```python
from build123d import *

# Parameters (mm, degrees)
SKETCH1_W                                            = 50
SKETCH1_H                                            = 10
SKETCH1_W_2                                          = 100
SKETCH1_H_2                                          = 200
BOSS_EXTRUDE1_DEPTH                                  = 100
CUT_EXTRUDE1_DEPTH                                   = 174.205080757
CUT_EXTRUDE1_DEPTH_BACK                              = 174.205080757
SKETCH7_W                                            = 80
SKETCH7_H                                            = 80
CUT_EXTRUDE2_DEPTH                                   = 100
SKETCH8_R                                            = 20
CUT_EXTRUDE3_DEPTH                                   = 20
CSK_FOR_M6_HEXAGON_LOBULAR_SOCKET_RAISED_D           = 6.6
CSK_FOR_M6_HEXAGON_LOBULAR_SOCKET_RAISED_CSINK_D     = 12.8
CSK_FOR_M6_HEXAGON_LOBULAR_SOCKET_RAISED_CSINK_ANGLE = 90
SKETCH13_W                                           = 20
SKETCH13_H                                           = 20
CUT_EXTRUDE4_DEPTH                                   = 10


with BuildPart() as part:
    # Sketch1 → Boss-Extrude1 (new body)
    with BuildSketch(Plane.XY):
        with Locations((-75, -95)):
            Rectangle(SKETCH1_W, SKETCH1_H)
        Rectangle(SKETCH1_W_2, SKETCH1_H_2)
        with Locations((75, -95)):
            Rectangle(SKETCH1_W, SKETCH1_H)
    extrude(amount=BOSS_EXTRUDE1_DEPTH)

    # Sketch5 → Cut-Extrude1 (cut, two sides: drawn at the far end of the back side and taken through both)
    with BuildSketch(Plane(origin=(0, 0, 0), x_dir=(0, 0, -1), z_dir=(1, 0, 0)).offset(-CUT_EXTRUDE1_DEPTH_BACK)):
        Polygon((-481.193494813, 352.459484715), (-100, 100), (0, 33.771302986), (381.193494813, -218.688181728), (886.112464242, 543.698807897), (23.725474617, 1114.84647434), align=None)
    extrude(amount=CUT_EXTRUDE1_DEPTH + CUT_EXTRUDE1_DEPTH_BACK, mode=Mode.SUBTRACT)

    # Sketch7 → Cut-Extrude2 (cut, symmetric)
    with BuildSketch(Plane(origin=(0, 0, 0), x_dir=(1, 0, 0), z_dir=(0, 1, 0))):
        with Locations((0, -50)):
            Rectangle(SKETCH7_W, SKETCH7_H)
    extrude(amount=CUT_EXTRUDE2_DEPTH, both=True, mode=Mode.SUBTRACT)

    # Sketch8 → Cut-Extrude3 (cut)
    with BuildSketch(Plane(origin=(0, 0, 0), x_dir=(-1, 0, 0), z_dir=(0, 0, -1))):
        with Locations((0, -40)):
            Circle(SKETCH8_R)
    extrude(amount=-CUT_EXTRUDE3_DEPTH, mode=Mode.SUBTRACT)

    # CSK for M6 Hexagon lobular socket raised CTSK head screws1 (through all)
    with Locations(Plane(origin=(0, -90, 0), x_dir=(1, 0, 0), z_dir=(0, 1, 0))):
        with Locations((-90, -10), (-90, -90), (90, -10), (90, -90)):
            CounterSinkHole(CSK_FOR_M6_HEXAGON_LOBULAR_SOCKET_RAISED_D / 2, CSK_FOR_M6_HEXAGON_LOBULAR_SOCKET_RAISED_CSINK_D / 2, counter_sink_angle=CSK_FOR_M6_HEXAGON_LOBULAR_SOCKET_RAISED_CSINK_ANGLE)

    # Sketch13 → Cut-Extrude4 (cut)
    with BuildSketch(Plane(origin=(50, 0, 0), x_dir=(0, 0, -1), z_dir=(1, 0, 0))):
        with Locations((-10, -80)):
            Rectangle(SKETCH13_W, SKETCH13_H)
    extrude(amount=-CUT_EXTRUDE4_DEPTH, mode=Mode.SUBTRACT)


solid = part.part
```
Verification items for the finished model (mm, model axes). A direction names the side the tool comes from. Coordinates: 2 decimals unless noted, no trailing zeros. Order: outer loops, then holes, each group sorted by start corner. A loop starts at its lowest first (then second) coordinate and runs counter-clockwise, first axis right, second up. Notation, with made-up numbers: (61.25, 72) -> (78.25, 72) arc R14 cw to (78.25, 88) -> close; hole circle Ø8 at (-10.75, 3.25). An arc over 180 degrees is marked (long way). Answer as CSV lines item,"result". Start each with the question number.
1) Release check for a two-part mould opening along X. For faces 5 (the face through (50, -17, 49)), 6 (the face through (-50, -17, 49)), 7 (the face through (43.74, 67.35, 50.7)), 8 (the face through (-87.57, -96.6, 87.77)) record: released by +X, released by -X, zero draft, split by the parting line, or undercut.
2) Set-up check for faces 1 (the face through (-93.29, -92.95, 88.96)), 2 (the face through (-1, -2, 90)), 3 (the face through (2.6, -20.17, 4.93)), 4 (the face through (45, -70, 10)): record each of +Z, -Z, +X, -X, +Y, -Y from which the full face is reachable in a straight line by a thin tool's end or side.
3) Material ranges on L1, parallel to Z at x = 90, y = -97.75; L2, parallel to Z at x = 33, y = -50.5; L3, parallel to X at y = 42.5, z = 49.5, recorded low to high. Write a range as [from, to].
4) Cross-section at A-A, the plane x = 0. Record the boundary of the cut face in (y, z).
5) Cross-section at D-D, the plane y = -40. Record the boundary of the cut face in (x, z), then the cut area to 3 significant figures.
6) Gauge pin test, flat ends, axial feed: pin 1 Ø7.5 at (x, z) = (90, 10) entering from +Y; pin 2 Ø5.5 at (x, z) = (-90, 10) entering from -Y; pin 3 Ø10 at (y, z) = (44, 86.5) entering from -X; pin 4 Ø10 at (y, z) = (13.5, 49.5) entering from +X. Record the tip position at first contact, or that the pin passes through.
7) Cross-section at B-B, the plane z = 37.5. Record the boundary of the cut face in (x, y).
8) Cross-section at C-C, the plane y = -8. Record the boundary of the cut face in (x, z), then the cut area to 3 significant figures.
Conclusion:
1,face 5,"released by +X"
1,face 6,"released by -X"
1,face 7,"zero draft"
1,face 8,"undercut"
2,face 1,"+Y"
2,face 2,"+Y, -Y"
2,face 3,"-Z"
2,face 4,"-Z, +X"
3,L1,"z = [0, 6.7], [13.3, 86.7], [93.3, 100]"
3,L2,"z = [0, 10], [90, 100]"
3,L3,"x = [-50, -40], [40, 50]"
4,outline,"(-100, 0) -> (-60, 0) -> (-60, 10) -> (-100, 10) -> close; (-100, 90) -> (93.38, 90) -> (100, 100) -> (-100, 100) -> close; (-20, 0) -> (33.77, 0) -> (40.39, 10) -> (-20, 10) -> close"
5,outline,"(-50, 0) -> (-20, 0) -> (-20, 10) -> (-40, 10) -> (-40, 90) -> (40, 90) -> (40, 10) -> (20, 10) -> (20, 0) -> (50, 0) -> (50, 100) -> (-50, 100) -> close"
5,area,"3,200 mm²"
6,pin 1,"stops at y = -92.65"
6,pin 2,"passes through"
6,pin 3,"stops at x = -50"
6,pin 4,"stops at x = 50"
7,outline,"(-100, -100) -> (-40, -100) -> (-40, 58.61) -> (-50, 58.61) -> (-50, -90) -> (-100, -90) -> close; (40, -100) -> (100, -100) -> (100, -90) -> (50, -90) -> (50, 58.61) -> (40, 58.61) -> close"
8,outline,"(-50, 0) -> (50, 0) -> (50, 100) -> (-50, 100) -> close; hole (-40, 10) -> (40, 10) -> (40, 90) -> (-40, 90) -> close"
8,area,"3,600 mm²"
